The drawing under review shows one solid part. Ordinate dimensions are in mm from its lowest x, y, z. A direction names the side the tool comes from. Round coordinates to 2 decimals unless told otherwise and drop trailing zeros. Write each loop counter-clockwise with the first axis right and the second up, starting at its lowest first coordinate (ties: lowest second). Pieces come first, ordered by that corner, then holes. Notation, with made-up numbers: (20, 41) -> (42, 41) arc R4 cw to (42, 46) -> close; hole circle Ø7 at (88.25, 10). An arc over 180 degrees is marked (long way). Answer in a Markdown table with one row per item.
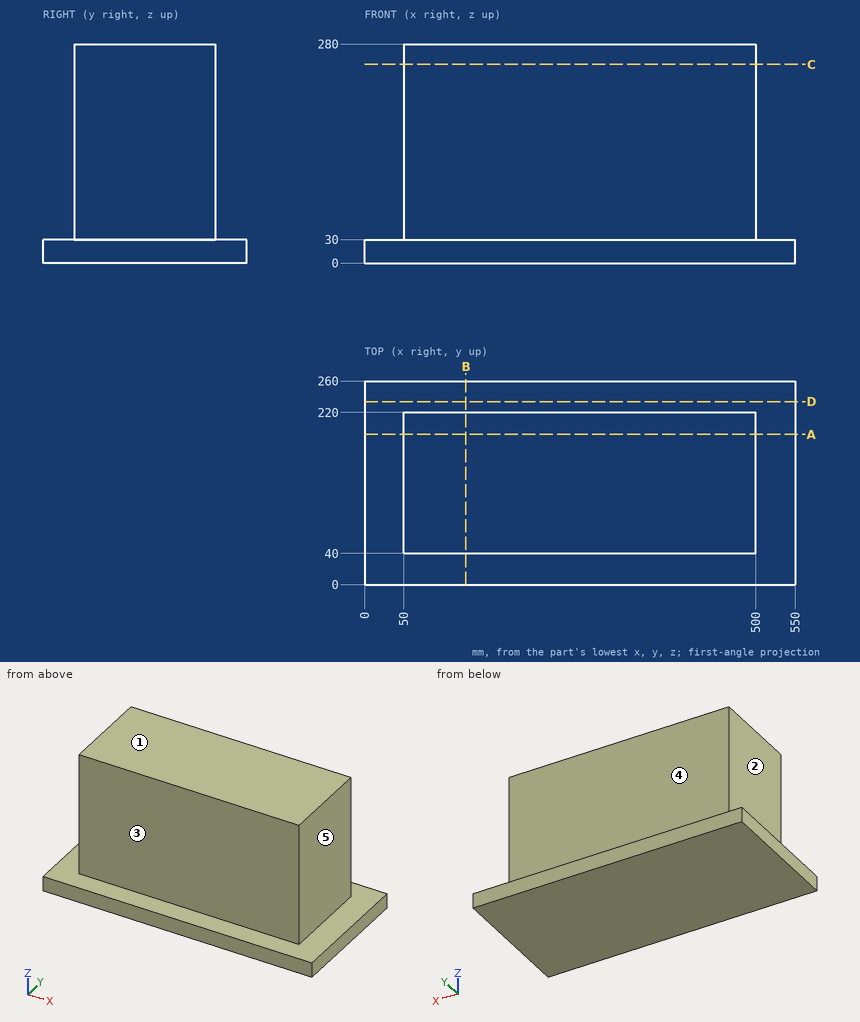
1) For line 1 (Y direction, x = 367.5, z = 48.5); line 2 (Z direction, x = 28.5, y = 224.5); line 3 (X direction, y = 203.5, z = 247), list the stretches that pass through material, from the lowest coordinate up. Write a range as [from, to].
Solved:
| item | result |
|---|---|
| line 1 | [40, 220] |
| line 2 | [0, 30] |
| line 3 | [50, 500] |
2) Consider section D-D on y = 234. State the section outline as (x, z) points, then the cut area to 3 significant figures.
Solved:
| item | result |
|---|---|
| outline | (0, 0) -> (550, 0) -> (550, 30) -> (0, 30) -> close |
| area | 16,500 mm² |
3) For the marked faces 1, 2, 3, 4 and 5, list the 3-axis set-ups (+Z, -Z, +X, -X, +Y, -Y) from which the entire face can be reached by the end or side of a thin tool; tool diameter is ignored.
Solved:
| item | result |
|---|---|
| face 1 | +Z, +X, -X, +Y, -Y |
| face 2 | +Z, -X, +Y, -Y |
| face 3 | +Z, +X, -X, -Y |
| face 4 | +Z, +X, -X, +Y |
| face 5 | +Z, +X, +Y, -Y |
4) Clearance check with flat-ended pins moving along their axes: pin 1 Ø3 at (x, z) = (220, 55.5) entering from +Y; pin 2 Ø12 at (x, z) = (146, 166) entering from -Y; pin 3 Ø5 at (y, z) = (148.5, 130.5) entering from -X. State where each tip first meets the part, or that it passes through.
Solved:
| item | result |
|---|---|
| pin 1 | y = 220 |
| pin 2 | y = 40 |
| pin 3 | x = 50 |
5) Consider section C-C on z = 254. State the section outline as (x, y) points.
Solved:
| item | result |
|---|---|
| outline | (50, 40) -> (500, 40) -> (500, 220) -> (50, 220) -> close |
6) Consider section B-B on x = 129.5. State the section outline as (y, z) points.
Solved:
| item | result |
|---|---|
| outline | (0, 0) -> (260, 0) -> (260, 30) -> (220, 30) -> (220, 280) -> (40, 280) -> (40, 30) -> (0, 30) -> close |
7) Consider section A-A on y = 192. State the section outline as (x, z) points.
Solved:
| item | result |
|---|---|
| outline | (0, 0) -> (550, 0) -> (550, 30) -> (500, 30) -> (500, 280) -> (50, 280) -> (50, 30) -> (0, 30) -> close |
